```python
from build123d import *

# Parameters (mm, degrees)
BASE_PLATE_SKETCH_W                      = 105
BASE_PLATE_SKETCH_H                      = 65
BASE_PLATE_DEPTH                         = 16
LOCATING_KEY_SKETCH_W                    = 31
LOCATING_KEY_SKETCH_H                    = 16
LOCATING_KEY_DEPTH                       = 105
MOUNTING_HOLES_DEPTH                     = 70.544949493
MOUNTING_HOLES_DEPTH_BACK                = 70.544949493
MOUNTING_HOLES_SKETCH_R                  = 7
INCLINED_CYLINDER_BOSS_REACH             = 71.545
BOSS_PROFILE_SKETCH_R                    = 15
BOSS_PROFILE_SKETCH_R_2                  = 10.5
INCLINED_CYLINDER_BOSS_DIRECTION_2_REACH = 71.545
BOSS_BORE_DEPTH                          = 70.544949493
BOSS_BORE_DEPTH_BACK                     = 70.544949493
BOSS_BORE_SKETCH_R                       = 10.5
BOSS_BLEND_FILLET_R5_R                   = 5


with BuildPart() as part:
    # Base Plate Sketch → Base Plate (new body)
    with BuildSketch(Plane(origin=(0, 0, 0), x_dir=(1, 0, 0), z_dir=(0, 1, 0))):
        Rectangle(BASE_PLATE_SKETCH_W, BASE_PLATE_SKETCH_H)
    extrude(amount=-BASE_PLATE_DEPTH)

    # Locating Key Sketch → Locating Key (add)
    with BuildSketch(Plane.ZY.offset(52.5)):
        with Locations((0, -24)):
            Rectangle(LOCATING_KEY_SKETCH_W, LOCATING_KEY_SKETCH_H)
    extrude(amount=-LOCATING_KEY_DEPTH)

    # Mounting Holes Sketch → Mounting Holes (cut, two sides: drawn at the far end of the back side and taken through both)
    with BuildSketch(Plane(origin=(0, 0, 0), x_dir=(1, 0, 0), z_dir=(0, 1, 0)).offset(-MOUNTING_HOLES_DEPTH_BACK)):
        with Locations(Location((-37.5, 0, 0), (0, 0, 270))):
            Circle(MOUNTING_HOLES_SKETCH_R)
        with Locations(Location((37.5, 0, 0), (0, 0, 270))):
            Circle(MOUNTING_HOLES_SKETCH_R)
    extrude(amount=MOUNTING_HOLES_DEPTH + MOUNTING_HOLES_DEPTH_BACK, mode=Mode.SUBTRACT)

    # Inclined Cylinder Boss: up to this plane
    inclined_cylinder_boss_end = Plane(origin=(-52.5, -16, 32.5), z_dir=(0, 0, 1))
    # Boss Profile Sketch → Inclined Cylinder Boss (add, up to the surface)
    with BuildSketch(Plane(origin=(0, 0, 0), x_dir=(0.819152044288991, 0, 0.5735764363510473), z_dir=(-0.5735764363510473, 0, 0.819152044288991)), mode=Mode.PRIVATE) as inclined_cylinder_boss_sk1:
        Circle(BOSS_PROFILE_SKETCH_R)
        Circle(BOSS_PROFILE_SKETCH_R_2, mode=Mode.SUBTRACT)
    inclined_cylinder_boss_tool1 = split(extrude(inclined_cylinder_boss_sk1.sketch, amount=INCLINED_CYLINDER_BOSS_REACH, mode=Mode.PRIVATE), bisect_by=inclined_cylinder_boss_end, keep=Keep.BOTH, mode=Mode.PRIVATE)
    add(inclined_cylinder_boss_tool1.solids().sort_by_distance((-11.939744, 0, -8.360299))[0])

    # Inclined Cylinder Boss direction 2: up to this plane
    inclined_cylinder_boss_direction_2_end = Plane(origin=(-52.5, -16, -32.5), z_dir=(0, 0, -1))
    # Boss Profile Sketch → Inclined Cylinder Boss direction 2 (add, up to the surface)
    with BuildSketch(Plane(origin=(0, 0, 0), x_dir=(0.819152044288991, 0, 0.5735764363510473), z_dir=(-0.5735764363510473, 0, 0.819152044288991)), mode=Mode.PRIVATE) as inclined_cylinder_boss_direction_2_sk1:
        Circle(BOSS_PROFILE_SKETCH_R)
        Circle(BOSS_PROFILE_SKETCH_R_2, mode=Mode.SUBTRACT)
    inclined_cylinder_boss_direction_2_tool1 = split(extrude(inclined_cylinder_boss_direction_2_sk1.sketch, amount=-INCLINED_CYLINDER_BOSS_DIRECTION_2_REACH, mode=Mode.PRIVATE), bisect_by=inclined_cylinder_boss_direction_2_end, keep=Keep.BOTH, mode=Mode.PRIVATE)
    add(inclined_cylinder_boss_direction_2_tool1.solids().sort_by_distance((-11.939744, 0, -8.360299))[0])

    # Boss Bore Sketch → Boss Bore (cut, two sides: drawn at the far end of the back side and taken through both)
    with BuildSketch(Plane(origin=(0, 0, 0), x_dir=(0.819152044288991, 0, 0.5735764363510473), z_dir=(-0.5735764363510473, 0, 0.819152044288991)).offset(-BOSS_BORE_DEPTH_BACK)):
        with Locations(Location((0, 0, 0), (0, 0, 180))):
            Circle(BOSS_BORE_SKETCH_R)
    extrude(amount=BOSS_BORE_DEPTH + BOSS_BORE_DEPTH_BACK, mode=Mode.SUBTRACT)

    # Boss Blend Fillet R5
    boss_blend_fillet_r5_edges = [part.edges().sort_by_distance(p)[0] for p in [
        (-18.311618831, 0, 0),
        (18.311618831, 0, 0),
    ]]
    fillet(boss_blend_fillet_r5_edges, radius=BOSS_BLEND_FILLET_R5_R)


solid = part.part
```
The model under review builds one solid part; all positions refer to its coordinate system, in mm. A direction names the side the tool comes from. Round coordinates to 2 decimals unless told otherwise and drop trailing zeros. Loops run counter-clockwise (first coordinate to the right, second up) from the corner with the lowest first, then second, coordinate; pieces in that order, holes last. Notation, with made-up numbers: M 62,71 L 86,71 A30 ccw 86,96 Z; hole C -27,-14.5 d2. An arc over 180 degrees is marked long. Put each result on its own line as item: value.
Q1. Consider section C-C, the plane z = 1. Count the separate pieces of the cut face and the enclosed holes in it, then the cut area to 3 significant figures.
Result set:
separate pieces: 3
enclosed holes: 1
area: 2,490 mm²
Q2. To check wall thickness, follow L1, parallel to X at y = -23, z = 0; L2, parallel to Z at x = 37.5, y = -18.5; L3, parallel to Z at x = 37, y = -15. State the ranges of each line that lie inside material, in increasing order.
Result set:
L1: x = -52.5 to -44.5, -30.5 to 30.5, 44.5 to 52.5
L2: z = -15.5 to -7, 7 to 15.5
L3: z = -32.5 to -6.98, 6.98 to 32.5
Q3. Machinability: for faces 4 (the flat face through (-1, -24, 15.5)), 5 (the flat face through (-33, 0, -8)), 6 (the flat face through (32, 0, 7)), which of the approach directions +Z, -Z, +X, -X, +Y, -Y give a long, thin tool a straight path to every point of the face, cutting with its end or side? Answer none if there is none.
Result set:
face 4: +Z, +X, -X, -Y
face 5: -Z, -X, +Y
face 6: +Z, +X, +Y
Q4. Mouldability with a two-part tool opening along Z and no side actions: class faces 1 (the cylindrical face through (-30.56, -16.22, -0.91)), 2 (the flat face through (-1, -32, 0)), 3 (the flat face through (-1, -24, -15.5)) as released by +Z, released by -Z, zero draft, split by the parting line, or undercut.
Result set:
face 1: undercut
face 2: zero draft
face 3: released by -Z
Q5. Consider section A-A, the plane y = 2.5. Give the boundary of the cut face in (x, z).
Result set:
outline: M -41.11,32.5 L 4.4,-32.5 L 10.31,-32.5 L -35.21,32.5 Z; M -10.31,32.5 L 35.21,-32.5 L 41.11,-32.5 L -4.4,32.5 Z
Q6. Consider section B-B, the plane y = -21.5. Give the boundary of the cut face in (x, z).
Result set:
outline: M -52.5,-15.5 L 52.5,-15.5 L 52.5,15.5 L -52.5,15.5 Z; hole C -37.5,0 d14; hole C 37.5,0 d14
Q7. For pin 1 (3 mm diameter, centred on x = 21.5, y = 8, fed in from +Z); pin 2 (12 mm diameter, centred on x = 31, y = 10, fed in from +Z); pin 3 (12 mm diameter, centred on y = 8, z = -9.5, fed in from +X), all flat-tipped, find the tip position at first contact; note any pin that passes through.
Result set:
pin 1: stops at z = -5.95
pin 2: stops at z = -13.71
pin 3: stops at x = 27.56
